Answer from the drawing. Dimensions are ordinates in mm from the lowest x, y and z of the part. Coordinates: 2 decimals unless noted, no trailing zeros. Write each loop counter-clockwise with the first axis right and the second up, starting at its lowest first coordinate (ties: lowest second). Pieces come first, ordered by that corner, then holes. Notation, with made-up numbers: M 34,32 L 82,32 A31 cw 82,65 Z; hole C 47,19 d8. An arc over 180 degrees is marked long. Put each result on its own line as item: value. Start each with the question number.
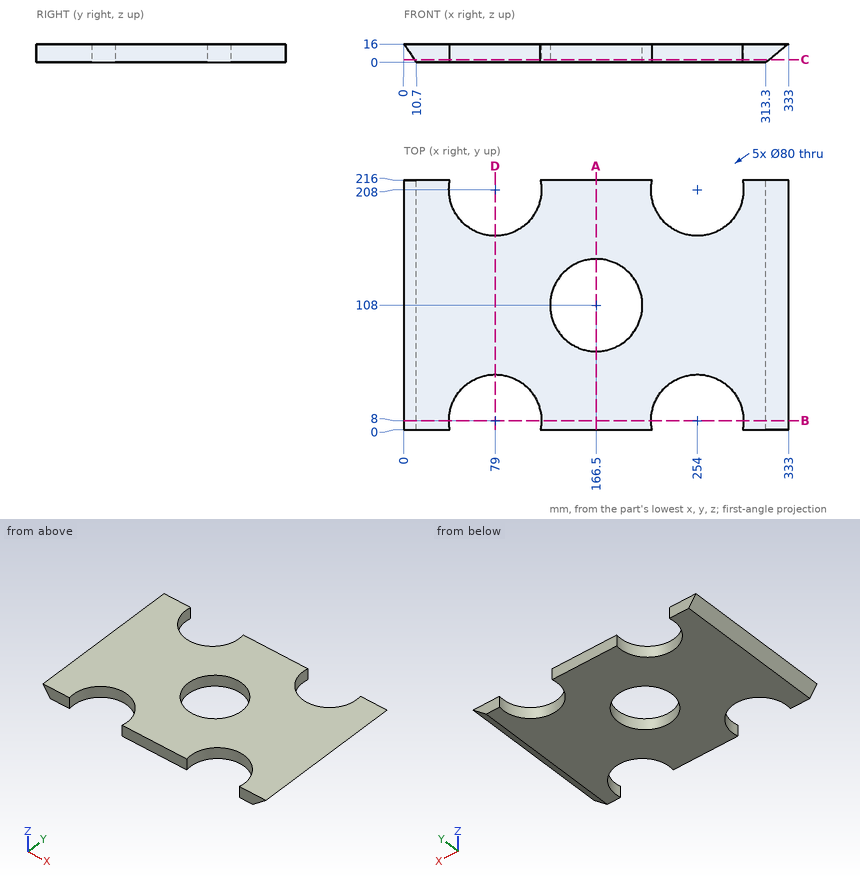
1) A cutting plane is placed at B-B on y = 8. Write down the section's boundary in (x, z), then the cut area to 3 significant figures.
2) A cutting plane is placed at C-C on z = 2.5. Write down the section's boundary in (x, y).
3) Straight lines are drawn through the part: probe 1 along X at (y, z) = (8, 12.25); probe 2 along X at (y, z) = (208, 11.75); probe 3 along Y at (x, z) = (254, 6.75). For each, find the intervals that lie inside material, in ascending order.
4) A cutting plane is placed at D-D on x = 79. Write down the section's boundary in (y, z).
5) A cutting plane is placed at A-A on x = 166.5. Write down the section's boundary in (y, z).
6) Given pin 1 Ø1.5 at (y, z) = (192, 9.5) entering from -X; pin 2 Ø1.5 at (x, z) = (277, 6) entering from +Y; pin 3 Ø12 at (x, y) = (249.5, 169) entering from +Z; pin 4 Ø2 at (y, z) = (37, 12.5) entering from +X, each flat-ended and moving along its own axis, determine where each tip first touches the part or whether it passes through.
Answers follow:
1. outline: M 0,16 L 10.7,0 L 39,0 L 39,16 Z; M 119,0 L 214,0 L 214,16 L 119,16 Z; M 294,0 L 313.3,0 L 333,16 L 294,16 Z
1. area: 2,520 mm²
2. outline: M 9.03,0 L 39.81,0 A40 cw long 118.19,0 L 214.81,0 A40 cw long 293.19,0 L 316.38,0 L 316.38,216 L 293.19,216 A40 cw long 214.81,216 L 118.19,216 A40 cw long 39.81,216 L 9.03,216 Z; hole C 166.5,108 d80
3. probe 1: x = 2.51 to 39, 119 to 214, 294 to 328.38
3. probe 2: x = 2.84 to 39, 119 to 214, 294 to 327.77
3. probe 3: y = 48 to 168
4. outline: M 48,0 L 168,0 L 168,16 L 48,16 Z
5. outline: M 0,0 L 68,0 L 68,16 L 0,16 Z; M 148,0 L 216,0 L 216,16 L 148,16 Z
6. pin 1: stops at x = 3.85
6. pin 2: stops at y = 175.81
6. pin 3: stops at z = 16
6. pin 4: stops at x = 329.92
